from build123d import *

# Parameters (mm, degrees)
EXTRUDE_972_DEPTH      = 0.5
EXTRUDE_972_DEPTH_BACK = 0.5
SKETCH_1_R             = 0.85


with BuildPart() as part:
    # 草图1 → Extrude 972 (new, two sides: drawn at the far end of the back side and taken through both)
    with BuildSketch(Plane.XY.offset(-EXTRUDE_972_DEPTH_BACK)):
        with BuildLine():
            Line((-1, -7.327151675), (-1, -10.95227248))
            ThreePointArc((-1, -10.95227248), (-3.005026441, -10.560805936), (-4.896301332, -9.788500055))
            ThreePointArc((-4.896301332, -9.788500055), (-4.964631615, -9.729422113), (-5, -9.64630588))
            Line((-5, -9.64630588), (-5.566746879, -6.432124609))
            ThreePointArc((-5.566746879, -6.432124609), (-5.619937096, -6.280010711), (-5.718749028, -6.152715625))
            ThreePointArc((-5.718749028, -6.152715625), (0, 8.4), (5.718749028, -6.152715625))
            ThreePointArc((5.718749028, -6.152715625), (5.619937096, -6.280010711), (5.566746879, -6.432124609))
            Line((5.566746879, -6.432124609), (5, -9.64630588))
            ThreePointArc((5, -9.64630588), (4.964631615, -9.729422113), (4.896301332, -9.788500055))
            ThreePointArc((4.896301332, -9.788500055), (3.005026441, -10.560805936), (1, -10.95227248))
            Line((1, -10.95227248), (1, -7.327151675))
            ThreePointArc((1, -7.327151675), (0, 6.4), (-1, -7.327151675))
        make_face()
        with Locations((-3, -8.666394553)):
            Circle(SKETCH_1_R, mode=Mode.SUBTRACT)
        with Locations(Location((3, -8.666394553, 0), (0, 0, 180))):
            Circle(SKETCH_1_R, mode=Mode.SUBTRACT)
    extrude(amount=EXTRUDE_972_DEPTH + EXTRUDE_972_DEPTH_BACK)


solid = part.part
Verification items for the finished model (mm, model axes). A direction names the side the tool comes from. Coordinates: 2 decimals unless noted, no trailing zeros. Order: outer loops, then holes, each group sorted by start corner. A loop starts at its lowest first (then second) coordinate and runs counter-clockwise, first axis right, second up.
1. Release check for a two-part mould opening along Y. For faces 1 (the face through (-3.184, -9.496, -0.007)), 2 (the face through (-0.281, 8.395, -0.007)), 3 (the face through (-2.98, -10.57, -0.01)) record: +Y half, -Y half, draft (parallel to the pull), parting line (faces both ways), or undercut.
Results found:
face 1: undercut
face 2: parting line
face 3: -Y half
2. Sectioned sample at A-A, the plane y = 2.25. Record the cut outline in (x, z).
Results found:
outline: (-8.09, -0.5) - (-6.33, -0.5) - (-6.33, 0.5) - (-8.09, 0.5) - close; (6.33, -0.5) - (8.09, -0.5) - (8.09, 0.5) - (6.33, 0.5) - close
3. Set-up check for faces 4 (the face through (3.032, -10.553, -0.007)), 5 (the face through (1, -9, 0)): record each of +Z, -Z, +X, -X, +Y, -Y from which the full face is reachable in a straight line by a thin tool's end or side.
Results found:
face 4: +Z, -Z, +X, -Y
face 5: +Z, -Z, -Y
4. Scan lines: line 1 (Y direction, x = 3, z = -0.05); line 2 (X direction, y = -9.25, z = -0.35); line 3 (X direction, y = -8.25, z = 0.3). Record each from-to range of solid material in increasing order.
Results found:
line 1: y = -10.56 to -9.52, -7.82 to -6.71, 5.71 to 7.85
line 2: x = -5.07 to -3.62, -2.38 to -1, 1 to 2.38, 3.62 to 5.07
line 3: x = -5.25 to -3.74, -2.26 to -1, 1 to 2.26, 3.74 to 5.25
5. Sectioned sample at C-C, the plane x = 3. Record the cut outline in (y, z).
Results found:
outline: (-10.56, -0.5) - (-9.52, -0.5) - (-9.52, 0.5) - (-10.56, 0.5) - close; (-7.82, -0.5) - (-6.71, -0.5) - (-6.71, 0.5) - (-7.82, 0.5) - close; (5.71, -0.5) - (7.85, -0.5) - (7.85, 0.5) - (5.71, 0.5) - close
6. Sectioned sample at B-B, the plane x = -4.25. Record the cut outline in (y, z), and give its area (3 significant figures).
Results found:
outline: (-10.1, -0.5) - (-5.94, -0.5) - (-5.94, 0.5) - (-10.1, 0.5) - close; (4.94, -0.5) - (7.25, -0.5) - (7.25, 0.5) - (4.94, 0.5) - close
area: 6.48 mm2
7. Sectioned sample at D-D, the plane z = 0.1. Record the cut outline in (x, y).
Results found:
outline: (-5.72, -6.15) arc R0.5 cw to (-5.57, -6.43) - (-5, -9.65) arc R0.2 ccw to (-4.9, -9.79) arc R10.5 ccw to (-1, -10.95) - (-1, -7.33) arc R6.9 cw (long way) to (1, -7.33) - (1, -10.95) arc R10.5 ccw to (4.9, -9.79) arc R0.2 ccw to (5, -9.65) - (5.57, -6.43) arc R0.5 cw to (5.72, -6.15) arc R8.4 ccw (long way) to start; hole circle Ø1.7 at (-3, -8.67); hole circle Ø1.7 at (3, -8.67)
8. Go/stop test with flat-tipped pins: pin 1 Ø1 at (x, y) = (3, -8.67) entering from -Z; pin 2 Ø6 at (x, y) = (2, 5) entering from +Z. Record where each tip stops, or that it passes through.
Results found:
pin 1: passes through
pin 2: stops at z = 0.5
